Work out the finished part from the listing and answer in its coordinate system (mm). A direction names the side the tool comes from. Coordinates: 2 decimals unless noted, no trailing zeros. Order: outer loops, then holes, each group sorted by start corner. A loop starts at its lowest first (then second) coordinate and runs counter-clockwise, first axis right, second up. Notation, with made-up numbers: (55.5, 71) -> (89.5, 71) arc R15 ccw to (89.5, 81) -> close; hole circle Ø10 at (29, -2). An arc over 180 degrees is marked (long way). Answer as CSV lines item,"result". Start each with the question number.
Item 1: Section C-C (x = -19) is taken. Write down the section's boundary in (y, z), then the cut area to 3 significant figures.
Item 2: Section B-B (x = -29) is taken. Write down the section's boundary in (y, z).
Item 3: Section A-A (z = 2.5) is taken. Write down the section's boundary in (x, y).
Item 4: Straight lines are drawn through the part: L1, parallel to X at y = 28.15, z = 17; L2, parallel to X at y = 30.4, z = 0.5; L3, parallel to Z at x = -26.5, y = 27.3. For each, find the intervals that lie inside material, in ascending order.
Item 5: Each of these flat-tipped pins is pushed along its axis until it touches: pin 1 Ø1 at (x, z) = (-22, 4.5) entering from -Y; pin 2 Ø6 at (x, z) = (-39.5, 4.5) entering from -Y; pin 3 Ø1.5 at (y, z) = (29.5, -7) entering from -X. Where does it stop, or does it pass through?
Item 6: Which of the six approach directions +Z, -Z, +X, -X, +Y, -Y give full straight-line access (tool end or side, diameter ignored) to faces 1 (the face through (-30.694, 26, 2)), 2 (the face through (-29.3, 29.31, -11.53)), 3 (the face through (-28.454, 30.282, 9.683)), 4 (the face through (-21.01, 30.28, 2.76)), 5 (the face through (-28, 25.799, 2))?
Item 7: Section D-D (z = 16) is taken. Write down the section's boundary in (x, y).
```python
from build123d import *

# Parameters (mm, degrees)
SKETCH1_W           = 5
SKETCH1_H           = 5
BOSS_EXTRUDE1_DEPTH = 5
SKETCH2_R           = 2
BOSS_EXTRUDE2_DEPTH = 13.5
SKETCH3_R           = 2
BOSS_EXTRUDE3_DEPTH = 13.5
SKETCH4_R           = 2
SKETCH4_R_2         = 1.5
CUT_EXTRUDE1_DEPTH  = 4
SKETCH5_R           = 2
SKETCH5_R_2         = 1.5
CUT_EXTRUDE2_DEPTH  = 4


with BuildPart() as part:
    # Sketch1 → Boss-Extrude1 (new body)
    with BuildSketch(Plane.XY):
        with Locations((-28.193643968, 28.298971706)):
            Rectangle(SKETCH1_W, SKETCH1_H)
    extrude(amount=BOSS_EXTRUDE1_DEPTH)

    # Sketch2 → Boss-Extrude2 (add)
    with BuildSketch(Plane.XY.offset(5)):
        with Locations((-28.193643968, 28.298971706)):
            Circle(SKETCH2_R)
    boss_extrude2 = extrude(amount=BOSS_EXTRUDE2_DEPTH)

    # Sketch3 → Boss-Extrude3 (add)
    with BuildSketch(Plane(origin=(-25.693643968, 0, 0), x_dir=(0, 0, -1), z_dir=(1, 0, 0))):
        with Locations((-2.5, 28.298971706)):
            Circle(SKETCH3_R)
    boss_extrude3 = extrude(amount=BOSS_EXTRUDE3_DEPTH)

    # Mirror1: Boss-Extrude2 across plane
    add(boss_extrude2.mirror(Plane(origin=(0, 0, 2.5), x_dir=(1, 0, 0), z_dir=(0, 0, -1))))

    # Mirror2: Boss-Extrude3 across plane
    add(boss_extrude3.mirror(Plane(origin=(-28.193643968, 0, 0), x_dir=(0, 0, 1), z_dir=(1, 0, 0))))

    # Sketch4 → Cut-Extrude1 (cut)
    with BuildSketch(Plane.XY.offset(18.5)):
        with Locations((-28.193643968, 28.298971706)):
            Circle(SKETCH4_R)
        with Locations((-28.193643968, 28.298971706)):
            Circle(SKETCH4_R_2, mode=Mode.SUBTRACT)
    cut_extrude1 = extrude(amount=-CUT_EXTRUDE1_DEPTH, mode=Mode.SUBTRACT)

    # Mirror3: Cut-Extrude1 across plane
    add(cut_extrude1.mirror(Plane(origin=(0, 0, 2.5), x_dir=(1, 0, 0), z_dir=(0, 0, -1))), mode=Mode.SUBTRACT)

    # Sketch5 → Cut-Extrude2 (cut)
    with BuildSketch(Plane.ZY.offset(44.193643968)):
        with Locations(Location((2.5, 28.298971706, 0), (0, 0, 180))):
            Circle(SKETCH5_R)
        with Locations((2.5, 28.298971706)):
            Circle(SKETCH5_R_2, mode=Mode.SUBTRACT)
    cut_extrude2 = extrude(amount=-CUT_EXTRUDE2_DEPTH, mode=Mode.SUBTRACT)

    # Mirror4: Cut-Extrude2 across plane
    add(cut_extrude2.mirror(Plane(origin=(-28.193643968, 0, 0), x_dir=(0, 0, 1), z_dir=(1, 0, 0))), mode=Mode.SUBTRACT)


solid = part.part
```
Checked values:
1,outline,"circle Ø4 at (28.3, 2.5)"
1,area,"12.6 mm^2"
2,outline,"(25.8, 0) -> (26.47, 0) -> (26.47, -9.5) -> (27.03, -9.5) -> (27.03, -13.5) -> (29.56, -13.5) -> (29.56, -9.5) -> (30.13, -9.5) -> (30.13, 0) -> (30.8, 0) -> (30.8, 5) -> (30.13, 5) -> (30.13, 14.5) -> (29.56, 14.5) -> (29.56, 18.5) -> (27.03, 18.5) -> (27.03, 14.5) -> (26.47, 14.5) -> (26.47, 5) -> (25.8, 5) -> close"
3,outline,"(-44.19, 26.8) -> (-40.19, 26.8) -> (-40.19, 26.3) -> (-30.69, 26.3) -> (-30.69, 25.8) -> (-25.69, 25.8) -> (-25.69, 26.3) -> (-16.19, 26.3) -> (-16.19, 26.8) -> (-12.19, 26.8) -> (-12.19, 29.8) -> (-16.19, 29.8) -> (-16.19, 30.3) -> (-25.69, 30.3) -> (-25.69, 30.8) -> (-30.69, 30.8) -> (-30.69, 30.3) -> (-40.19, 30.3) -> (-40.19, 29.8) -> (-44.19, 29.8) -> close"
4,L1,"x = -29.69 to -26.7"
4,L2,"x = -30.69 to -25.69"
4,L3,"z = -9.5 to 14.5"
5,pin 1,"stops at y = 26.98"
5,pin 2,"stops at y = 26.3"
5,pin 3,"stops at x = -30.14"
6,face 1,"-X"
6,face 2,"-Z"
6,face 3,"+Z"
6,face 4,"+X"
6,face 5,"+Z, -Z, +X, -X, -Y"
7,outline,"circle Ø3 at (-28.19, 28.3)"
